Source: CAD feature listing. Evaluate the final solid. Frame: model axes, mm. A direction names the side the tool comes from. Round coordinates to 2 decimals unless told otherwise and drop trailing zeros. Loops run counter-clockwise (first coordinate to the right, second up) from the corner with the lowest first, then second, coordinate; pieces in that order, holes last. Notation, with made-up numbers: (66.5, -26.5) -> (125.5, -26.5) arc R25 ccw to (125.5, 8.5) -> close; hole circle Ø10 at (82, -20.75). An arc over 180 degrees is marked (long way). Write item = value, one per line.
from build123d import *

# Parameters (mm, degrees)
EXTRUDE_1_DEPTH = 7.5


with BuildPart() as part:
    # 草图1 → 凸台-拉伸1 (new, symmetric)
    with BuildSketch(Plane.XY):
        with BuildLine():
            Line((0, 14.17), (852.5, 14.17))
            ThreePointArc((852.5, 14.17), (866.67, 0), (852.5, -14.17))
            Line((852.5, -14.17), (0, -14.17))
            ThreePointArc((0, -14.17), (-14.17, 0), (0, 14.17))
        make_face()
        with BuildLine():
            Line((0, 12.99), (852.5, 12.99))
            ThreePointArc((852.5, 12.99), (865.49, 0), (852.5, -12.99))
            Line((852.5, -12.99), (0, -12.99))
            ThreePointArc((0, -12.99), (-12.99, 0), (0, 12.99))
        make_face(mode=Mode.SUBTRACT)
    extrude(amount=EXTRUDE_1_DEPTH, both=True)


solid = part.part
1. Section query B-B (x = 504). Return the cut outline in (y, z), then the cut area to 3 significant figures.
Evaluation:
outline = (-14.17, -7.5) -> (-12.99, -7.5) -> (-12.99, 7.5) -> (-14.17, 7.5) -> close; (12.99, -7.5) -> (14.17, -7.5) -> (14.17, 7.5) -> (12.99, 7.5) -> close
area = 35.4 mm²
2. Section query C-C (z = -2.75). Return the cut outline in (x, y), then the cut area to 3 significant figures.
Evaluation:
outline = (0, -14.17) -> (852.5, -14.17) arc R14.17 ccw to (852.5, 14.17) -> (0, 14.17) arc R14.17 ccw to start; hole (0, -12.99) -> (852.5, -12.99) arc R12.99 ccw to (852.5, 12.99) -> (0, 12.99) arc R12.99 ccw to start
area = 2,110 mm²
3. Section query A-A (y = 0). Return the cut outline in (x, z), then the cut area to 3 significant figures.
Evaluation:
outline = (-14.17, -7.5) -> (-12.99, -7.5) -> (-12.99, 7.5) -> (-14.17, 7.5) -> close; (865.49, -7.5) -> (866.67, -7.5) -> (866.67, 7.5) -> (865.49, 7.5) -> close
area = 35.4 mm²
4. Contact query for a flat-ended pin moving along its axis: pin 1 Ø1 at (y, z) = (9, -2) entering from -X. Output: stop coordinate, or through.
Evaluation:
pin_1 = -11.34
5. Line query: probe 1 along Y at (x, z) = (193.5, 0); probe 2 along X at (y, z) = (0.5, 5.5); probe 3 along X at (y, z) = (-0.75, 2.75). Output: solid intervals per line, ascending. Write a range as from..to.
Evaluation:
probe_1 = -14.17..-12.99, 12.99..14.17
probe_2 = -14.16..-12.98, 865.48..866.66
probe_3 = -14.15..-12.97, 865.47..866.65
6. Mould query, pull axis X, two halves, no side actions, for faces 1 (the face through (428, 14, -7.5)), 2 (the face through (420, 12.99, 0)), 3 (the face through (-12.987, -0.286, 0.105)), 4 (the face through (-14.167, -0.312, 0.105)). Classes: released by +X, released by -X, zero draft, split by the parting line, or undercut.
Evaluation:
face_1 = zero draft
face_2 = undercut
face_3 = undercut
face_4 = released by -X
7. Set-up query: faces 5 (the face through (866.667, 0.312, 0.105)), 6 (the face through (432, -12.99, 0)). Return all of +Z, -Z, +X, -X, +Y, -Y with unobstructed straight access to the full face (end or side cutting, diameter ignored); none if empty.
Evaluation:
face_5 = +Z, -Z, +X
face_6 = +Z, -Z
